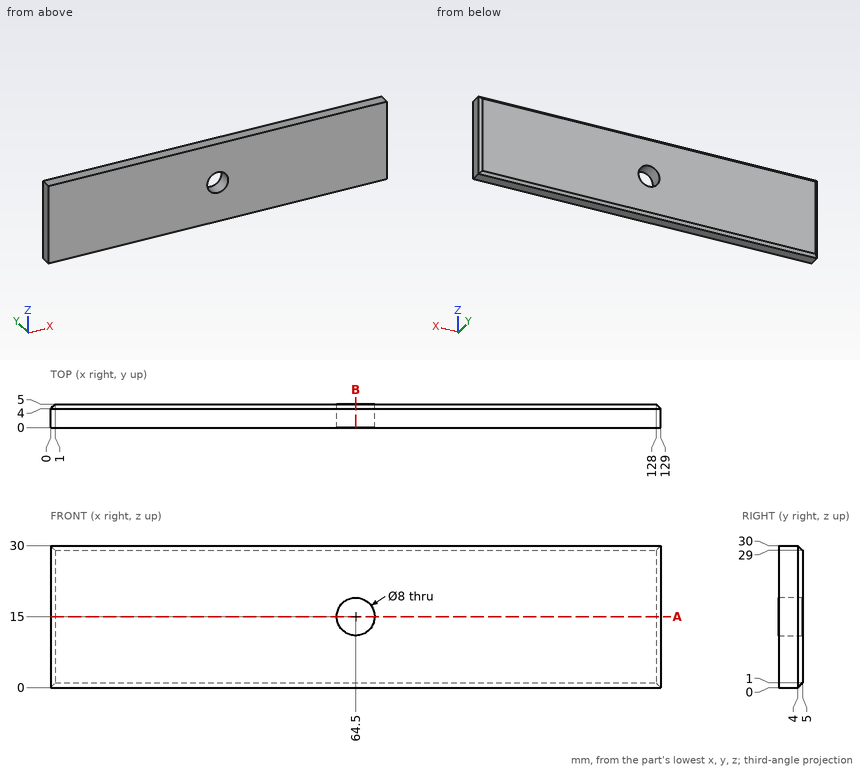
Check sheet for the drawn part. Datum: minimum x, y, z corner. Units: mm. Give positions to 0.01 mm unless a question says otherwise; leave off trailing zeros. Loops run counter-clockwise (first coordinate to the right, second up) from the corner with the lowest first, then second, coordinate; pieces in that order, holes last. Notation, with made-up numbers: (-13.5, 18) - (25.5, 18) arc R17 ccw to (25.5, 24) - close; hole circle Ø4 at (18.25, 14.5). An arc over 180 degrees is marked (long way). Write each question's results on one line, items separated by ' | '.
1) Material ranges on L1, parallel to X at y = 1.2, z = 15; L2, parallel to X at y = 3.95, z = 18; L3, parallel to Z at x = 121, y = 4.1, recorded low to high. Write a range as from..to.
Solution:
L1: 0..60.5, 68.5..129 | L2: 0..61.85, 67.15..129 | L3: 0.1..29.9
2) Sectioned sample at B-B on x = 64.5. Record the boundary of the cut face in (y, z), plus the area to 3 significant figures.
Solution:
outline: (0, 0) - (4, 0) - (5, 1) - (5, 11) - (0, 11) - close; (0, 19) - (5, 19) - (5, 29) - (4, 30) - (0, 30) - close | area: 109 mm2
3) Sectioned sample at A-A on z = 15. Record the boundary of the cut face in (x, y), plus the area to 3 significant figures.
Solution:
outline: (0, 0) - (60.5, 0) - (60.5, 5) - (1, 5) - (0, 4) - close; (68.5, 0) - (129, 0) - (129, 4) - (128, 5) - (68.5, 5) - close | area: 604 mm2
